The figure shows three views and two pictorial views of one solid part (mm, origin at its lowest corner). Answer the questions. A direction names the side the tool comes from. Coordinates: 2 decimals unless noted, no trailing zeros. Loops run counter-clockwise (first coordinate to the right, second up) from the corner with the lowest first, then second, coordinate; pieces in that order, holes last.
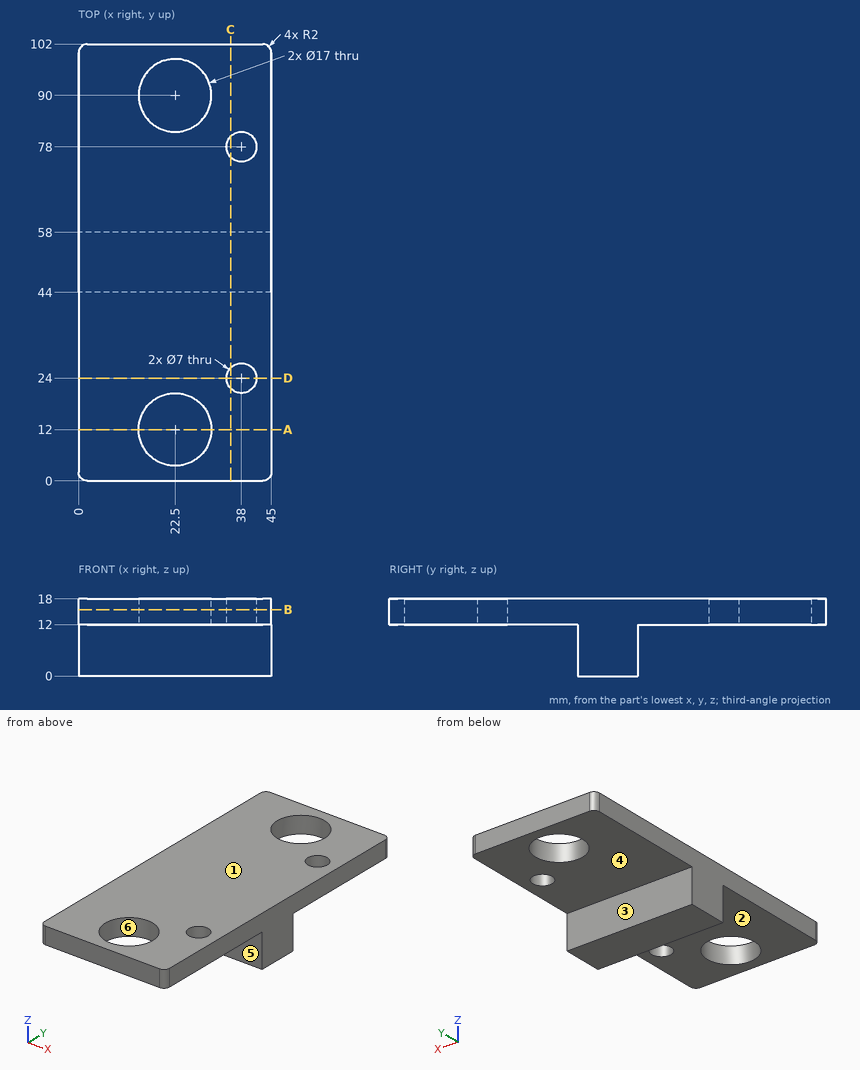
Q1. A cutting plane is placed at A-A (y = 12). Give the vertices of the cut face in (x, z).
Findings below:
outline: (0, 12) - (14, 12) - (14, 18) - (0, 18) - close; (31, 12) - (45, 12) - (45, 18) - (31, 18) - close
Q2. Determine the mould class of the marked faces 3, 4, 5 and 6 for opening direction Y: +Y half, -Y half, draft (parallel to the pull), parting line (faces both ways), or undercut.
Findings below:
face 3: +Y half
face 4: draft
face 5: -Y half
face 6: undercut
Q3. A cutting plane is placed at C-C (x = 35.5). Give the vertices of the cut face in (y, z).
Findings below:
outline: (0, 12) - (21.55, 12) - (21.55, 18) - (0, 18) - close; (26.45, 12) - (44, 12) - (44, 0) - (58, 0) - (58, 12) - (75.55, 12) - (75.55, 18) - (26.45, 18) - close; (80.45, 12) - (102, 12) - (102, 18) - (80.45, 18) - close
Q4. Which of the six approach directions +Z, -Z, +X, -X, +Y, -Y give full straight-line access (tool end or side, diameter ignored) to the marked faces 1 and 2?
Findings below:
face 1: +Z, +X, -X, +Y, -Y
face 2: -Z, +X, -X, -Y
Q5. A cutting plane is placed at D-D (y = 24). Give the vertices of the cut face in (x, z), then the cut area to 3 significant figures.
Findings below:
outline: (0, 12) - (34.5, 12) - (34.5, 18) - (0, 18) - close; (41.5, 12) - (45, 12) - (45, 18) - (41.5, 18) - close
area: 228 mm2
Q6. Flat-ended cylindrical pins translate along their axes: pin 1 Ø5 at (x, z) = (38, 7.5) entering from +Y; pin 2 Ø6 at (x, z) = (9.5, 2) entering from -Y; pin 3 Ø1 at (x, y) = (35.5, 86) entering from -Z. Find the tip coordinate at first contact, or state that the pin passes through.
Findings below:
pin 1: stops at y = 58
pin 2: stops at y = 44
pin 3: stops at z = 12
Q7. A cutting plane is placed at B-B (z = 15.5). Give the vertices of the cut face in (x, y), then the cut area to 3 significant figures.
Findings below:
outline: (0, 2) arc R2 ccw to (2, 0) - (43, 0) arc R2 ccw to (45, 2) - (45, 100) arc R2 ccw to (43, 102) - (2, 102) arc R2 ccw to (0, 100) - close; hole circle Ø17 at (22.5, 12); hole circle Ø17 at (22.5, 90); hole circle Ø7 at (38, 24); hole circle Ø7 at (38, 78)
area: 4,060 mm2
Q8. Straight lines are drawn through the part: probe 1 along Y at (x, z) = (22.5, 13.65); probe 2 along Y at (x, z) = (38, 16.4); probe 3 along Z at (x, y) = (29, 34). For each, find the intervals that lie inside material, in ascending order.
Findings below:
probe 1: y = 0 to 3.5, 20.5 to 81.5, 98.5 to 102
probe 2: y = 0 to 20.5, 27.5 to 74.5, 81.5 to 102
probe 3: z = 12 to 18
